from build123d import *

# Parameters (mm, degrees)
SKETCH_1_R      = 6
SKETCH_1_R_2    = 4
EXTRUDE_1_DEPTH = 4
CHAMFER_1_SIZE  = 0.3


with BuildPart() as part:
    # 草图1 → 凸台-拉伸1 (new, symmetric)
    with BuildSketch(Plane.XY):
        Circle(SKETCH_1_R)
        Circle(SKETCH_1_R_2, mode=Mode.SUBTRACT)
    extrude(amount=EXTRUDE_1_DEPTH, both=True)

    # 倒角1
    chamfer_1_edges = [part.edges().sort_by_distance(p)[0] for p in [
        (-6, 0, -4),
        (-6, 0, 4),
        (-4, 0, -4),
        (-4, 0, 4),
    ]]
    chamfer(chamfer_1_edges, length=CHAMFER_1_SIZE)


solid = part.part
Can you work these out from the model? Positions are in its coordinate system, mm. Give positions to 0.01 mm unless a question says otherwise; leave off trailing zeros. Loops run counter-clockwise (first coordinate to the right, second up) from the corner with the lowest first, then second, coordinate; pieces in that order, holes last. Notation, with made-up numbers: (63, 22) -> (105, 22) arc R16 ccw to (105, 32) -> close; hole circle Ø1 at (63, 69). An arc over 180 degrees is marked (long way). Use one line per item in the form item = value.
1) If we section it at A-A (y = 0): Please give me the cut outline in (x, z).
Answers:
outline = (-6, -3.7) -> (-5.7, -4) -> (-4.3, -4) -> (-4, -3.7) -> (-4, 3.7) -> (-4.3, 4) -> (-5.7, 4) -> (-6, 3.7) -> close; (4, -3.7) -> (4.3, -4) -> (5.7, -4) -> (6, -3.7) -> (6, 3.7) -> (5.7, 4) -> (4.3, 4) -> (4, 3.7) -> close
2) We'd pull the mould along Y, two halves only. Please class faces 1 (the face through (-0.867, -3.905, -0.052)), 2 (the face through (2, 4, 4)), 3 (the face through (-6, 0, 0)): released by +Y, released by -Y, zero draft, split by the parting line, or undercut.
Answers:
face_1 = undercut
face_2 = zero draft
face_3 = split by the parting line
3) I need wall thicknesses on line 1 along Y through (x, z) = (0, -1.5); line 2 along X through (y, z) = (-3, 0.25); line 3 along X through (y, z) = (-2, -3). Which ranges of each line are inside material? Lowest first, please.
Answers:
line_1 = -6 to -4, 4 to 6
line_2 = -5.2 to -2.65, 2.65 to 5.2
line_3 = -5.66 to -3.46, 3.46 to 5.66
4) Will these pins go through, and if not, where does the flat tip stop? pin 1 (3 mm diameter, centred on x = 2, z = 1.5, fed in from -Y); pin 2 (1 mm diameter, centred on y = 4.5, z = -1, fed in from -X); pin 3 (2 mm diameter, centred on x = -2.5, y = 0.5, fed in from +Z); pin 4 (1.5 mm diameter, centred on x = -3.5, z = 2.5, fed in from +Y).
Answers:
pin_1 = -5.98
pin_2 = -4.47
pin_3 = through
pin_4 = 5.33
5) If we section it at C-C (z = 1.25): Please give me the cut outline in (x, y).
Answers:
outline = circle Ø12 at (0, 0); hole circle Ø8 at (0, 0)
